For this review, take the finished solid that the model builds, in its own axes (mm). A direction names the side the tool comes from. Give positions to 0.01 mm unless a question says otherwise; leave off trailing zeros. Order: outer loops, then holes, each group sorted by start corner. A loop starts at its lowest first (then second) coordinate and runs counter-clockwise, first axis right, second up. Notation, with made-up numbers: (5.5, 4.5) -> (58.5, 4.5) arc R19 ccw to (58.5, 17.5) -> close; hole circle Ø6 at (79.5, 0). An arc over 180 degrees is marked (long way). Return JSON: item names as keys, results as strings. Group by question number.
1) Add section A-A (z = -44.5). Give the boundary of the cut face in (x, y), then the cut area to 3 significant figures.
2) Add section B-B (x = 55.5). Give the boundary of the cut face in (y, z), then the cut area to 3 significant figures.
3) Insertion check: P1, Ø1, axis at x = 30.5, z = -31, coming from the +Y side; P2, Ø12, axis at y = 56.5, z = -36.5, coming from the +X side; P3, Ø8, axis at x = 59, z = 107, coming from the -Y side. Each pin has a flat end and moves straight along its axis. Give the tip position at first contact, or say it passes through.
4) For faces 1 (the face through (10, 45, 3)), 2 (the face through (3, 75, 3)), list the 3-axis set-ups (+Z, -Z, +X, -X, +Y, -Y) from which the entire face can be reached by the end or side of a thin tool; tool diameter is ignored.
5) To check wall thickness, follow line 1 along X through (y, z) = (7, -93); line 2 along X through (y, z) = (60, -97). State the ranges of each line that lie inside material, in increasing order.
from build123d import *

# Parameters (mm, degrees)
BOSS_EXTRUDE1_DEPTH = 179.05


with BuildPart() as part:
    # Sketch1 → Boss-Extrude1 (new, symmetric)
    with BuildSketch(Plane.XY):
        with BuildLine():
            Line((0, 75), (0, 0))
            Line((0, 0), (75, 0))
            Line((75, 0), (75, 6.5))
            ThreePointArc((75, 6.5), (73.974873734, 8.974873734), (71.5, 10))
            Line((71.5, 10), (19, 10))
            ThreePointArc((19, 10), (12.636038969, 12.636038969), (10, 19))
            Line((10, 19), (10, 71.5))
            ThreePointArc((10, 71.5), (8.974873734, 73.974873734), (6.5, 75))
            Line((6.5, 75), (0, 75))
        make_face()
    extrude(amount=BOSS_EXTRUDE1_DEPTH, both=True)


solid = part.part
Evaluation:
{
 "1": {"outline": "(0, 0) -> (75, 0) -> (75, 6.5) arc R3.5 ccw to (71.5, 10) -> (19, 10) arc R9 cw to (10, 19) -> (10, 71.5) arc R3.5 ccw to (6.5, 75) -> (0, 75) -> close", "area": "1,410 mm^2"},
 "2": {"outline": "(0, -179.05) -> (10, -179.05) -> (10, 179.05) -> (0, 179.05) -> close", "area": "3,580 mm^2"},
 "3": {"P1": "y = 10", "P2": "x = 10", "P3": "y = 0"},
 "4": {"face 1": "+Z, -Z, +X, +Y", "face 2": "+Z, -Z, +X, -X, +Y"},
 "5": {"line 1": "0 to 74.96", "line 2": "0 to 10"}
}
